Part model, mm, in its own coordinate system. A direction names the side the tool comes from. Round coordinates to 2 decimals unless told otherwise and drop trailing zeros. Write each loop counter-clockwise with the first axis right and the second up, starting at its lowest first coordinate (ties: lowest second). Pieces come first, ordered by that corner, then holes. Notation, with made-up numbers: M 12.25,76 L 32.25,76 A9 cw 32.25,82 Z; hole C 22,-18 d3. An arc over 180 degrees is marked long. Answer as a JSON object with one key per item and string values. Group by question number.
1. Band-saw the part on B-B, the plane y = -16. Write the cut outline in (x, z).
2. Which spindle directions (+Z, -Z, +X, -X, +Y, -Y) get a long thin tool onto all of the face, cutting with end or side? Do faces 1 (the face through (3, -90, -60)), 2 (the face through (3, -10, -25)). Say none if no direction does.
3. Two-plate mould, pull along Z, no slides. Class faces 3 (the face through (3, 10, -30)), 4 (the face through (2.96, 6.99, -67.15)), 5 (the face through (2.958, -3.905, 0.867)): +Z half, -Z half, draft (parallel to the pull), parting line (faces both ways), or undercut.
4. Band-saw the part on C-C, the plane z = -13. Write the cut outline in (x, y), plus the area to 3 significant figures.
5. Band-saw the part on A-A, the plane x = 3.45. Write the cut outline in (y, z).
6. Drill centre lines: line 1 (Y direction, x = 1.65, z = -60); line 2 (Y direction, x = 1.2, z = -63); line 3 (Y direction, x = 2.3, z = -13.5). Where is each one in solid material? Low to high. Write a range as from..to.
7. Drop flat-ended pins along their axis: pin 1 (5 mm diameter, centred on y = -9.5, z = -12.5, fed in from -X); pin 2 (3 mm diameter, centred on x = 3.5, y = -4.5, fed in from +Z); pin 3 (1.5 mm diameter, centred on x = 3, y = -20, fed in from +Z); pin 4 (1.8 mm diameter, centred on x = 4, z = -31, fed in from -Y). Give the stop position or say it passes through.
from build123d import *

# Parameters (mm, degrees)
SKETCH1_R           = 4
BOSS_EXTRUDE1_DEPTH = 6


with BuildPart() as part:
    # Sketch1 → Boss-Extrude1 (new body)
    # profile 1 of 3: a face of its own
    with BuildSketch(Plane(origin=(0, 0, 0), x_dir=(0, 0, -1), z_dir=(1, 0, 0))):
        with BuildLine():
            Line((60, 10), (0, 10))
            ThreePointArc((0, 10), (-10, 0), (0, -10))
            Line((0, -10), (50, -10))
            Line((50, -10), (50, 0))
            ThreePointArc((50, 0), (52.928932188, 7.071067812), (60, 10))
        make_face()
        Circle(SKETCH1_R, mode=Mode.SUBTRACT)
    # profile 2 of 3: a face of its own
    with BuildSketch(Plane(origin=(0, 0, 0), x_dir=(0, 0, -1), z_dir=(1, 0, 0))):
        with BuildLine():
            ThreePointArc((70, 0), (67.071067812, 7.071067812), (60, 10))
            ThreePointArc((60, 10), (52.928932188, 7.071067812), (50, 0))
            Line((50, 0), (50, -10))
            Line((50, -10), (60, -10))
            ThreePointArc((60, -10), (67.071067812, -7.071067812), (70, 0))
        make_face()
        with Locations((60, 0)):
            Circle(SKETCH1_R, mode=Mode.SUBTRACT)
    # profile 3 of 3: a face of its own
    with BuildSketch(Plane(origin=(0, 0, 0), x_dir=(0, 0, -1), z_dir=(1, 0, 0))):
        with BuildLine():
            Line((70, -80), (70, 0))
            ThreePointArc((70, 0), (67.071067812, -7.071067812), (60, -10))
            Line((60, -10), (50, -10))
            Line((50, -10), (50, -80))
            ThreePointArc((50, -80), (60, -90), (70, -80))
        make_face()
        with Locations((60, -80)):
            Circle(SKETCH1_R, mode=Mode.SUBTRACT)
    extrude(amount=BOSS_EXTRUDE1_DEPTH)


solid = part.part
Worked answers:
{
 "1": {"outline": "M 0,-70 L 6,-70 L 6,-50 L 0,-50 Z"},
 "2": {"face 1": "+X, -X, -Y", "face 2": "+Z, +X, -X, -Y"},
 "3": {"face 3": "draft", "face 4": "-Z half", "face 5": "undercut"},
 "4": {"outline": "M 0,-10 L 6,-10 L 6,10 L 0,10 Z", "area": "120 mm^2"},
 "5": {"outline": "M -80,-70 L 0,-70 A10 ccw 10,-60 L 10,0 A10 ccw -10,0 L -10,-50 L -80,-50 A10 ccw Z; hole C -80,-60 d8; hole C 0,-60 d8; hole C 0,0 d8"},
 "6": {"line 1": "y = -90..-84, -76..-4, 4..10", "line 2": "y = -89.54..-82.65, -77.35..-2.65, 2.65..9.54", "line 3": "y = -10..10"},
 "7": {"pin 1": "stops at x = 0", "pin 2": "stops at z = 9.54", "pin 3": "stops at z = -50", "pin 4": "stops at y = -10"}
}
